from build123d import *

# Parameters (mm, degrees)
CUT_EXTRUDE_1_DEPTH      = 60.622226572
CUT_EXTRUDE_1_DEPTH_BACK = 60.622226572


with BuildPart() as part:
    # 扫描2: sweep along a path in Sketch 203
    with BuildLine(Plane.XY) as sweep_2_path:
        Line((55.4, 2.3), (5.4, 2.3))
        ThreePointArc((5.4, 2.3), (4.267859381, 2.531061156), (3.316806967, 3.187285922))
        ThreePointArc((3.316806967, 3.187285922), (-4.6, 0), (3.316806967, -3.187285922))
        ThreePointArc((3.316806967, -3.187285922), (4.267859381, -2.531061156), (5.4, -2.3))
        Line((5.4, -2.3), (59.4, -2.3))
    # 草图2 → 扫描2 (sweep)
    with BuildSketch(Plane(origin=(55.4, 2.3, 0), x_dir=(0, 0, 1), z_dir=(-1, 0, 0))):
        with BuildLine():
            Line((-2.299978261, -2.29), (2.299978261, -2.29))
            ThreePointArc((2.299978261, -2.29), (0, 0), (-2.299978261, -2.29))
        make_face()
    sweep(path=sweep_2_path.line)

    # 草图3 → 切除-拉伸1 (cut, two sides: drawn at the far end of the back side and taken through both)
    with BuildSketch(Plane.XY.offset(-CUT_EXTRUDE_1_DEPTH_BACK)):
        Polygon((55.4, 1.145), (53.76113083, 2.3), (59.41, 2.3), (59.41, -2.3), (57.754128755, -2.3), (59.4, -1.155), (57.76113083, 0), (53.754128755, 0), align=None)
    extrude(amount=CUT_EXTRUDE_1_DEPTH + CUT_EXTRUDE_1_DEPTH_BACK, mode=Mode.SUBTRACT)


solid = part.part
Read the model definition and answer for the solid it produces. Units are mm, in the model's axes. A direction names the side the tool comes from. Coordinates: 2 decimals unless noted, no trailing zeros. Loops run counter-clockwise (first coordinate to the right, second up) from the corner with the lowest first, then second, coordinate; pieces in that order, holes last.
Q1. The part is cut by section A-A on x = 15. Write down the section's boundary in (y, z), and give its area (3 significant figures).
Q2. Each of these flat-tipped pins is pushed along its axis until it touches: pin 1 Ø1 at (x, y) = (38, 1) entering from +Z (3 decimals); pin 2 Ø2 at (x, y) = (25.5, 2) entering from +Z; pin 3 Ø2 at (x, z) = (41.5, 1.5) entering from +Y (3 decimals). Where does it stop, or does it pass through?
Q3. Which of the six approach directions +Z, -Z, +X, -X, +Y, -Y give full straight-line access (tool end or side, diameter ignored) to faces 4 (the face through (32.78, -2.3, 0.05)), 5 (the face through (58.6, -0.59, -0.03))?
Q4. The mould has two halves that part along X. Classify faces 1 (the face through (54.77, 1.59, -0.03)), 2 (the face through (30.05, 2.3, 0.05)), 3 (the face through (3.4, 0.41, 0.03)): +X half, -X half, draft (parallel to the pull), parting line (faces both ways), or undercut.
Q5. Consider probe 1 along Y at (x, z) = (0, 0.1); probe 2 along Y at (x, z) = (0, -0.85); probe 3 along X at (y, z) = (-0.5, 1.2). Determine where each line is inside the solid, lowest interval first.
Results below:
1. outline: (-0.01, -2.3) - (-0.01, 2.3) arc R2.3 ccw to start; (0.01, -2.3) arc R2.3 ccw to (0.01, 2.3) - close
1. area: 16.5 mm2
2. pin 1: stops at z = 2.245
2. pin 2: stops at z = 2.07
2. pin 3: stops at y = 2.245
3. face 4: +X, -Y
3. face 5: +Z, -Z, +X, +Y
4. face 1: +X half
4. face 2: draft
4. face 3: undercut
5. probe 1: y = -4.6 to -2.31, 2.31 to 4.6
5. probe 2: y = -4.44 to -2.31, 2.31 to 4.44
5. probe 3: x = -4.23 to -2.26, 3.2 to 58.47
